The model under review builds one solid part; all positions refer to its coordinate system, in mm. Face numbers are marked on the shaded views. A direction names the side the tool comes from. Give positions to 0.01 mm unless a question says otherwise; leave off trailing zeros. Loops run counter-clockwise (first coordinate to the right, second up) from the corner with the lowest first, then second, coordinate; pieces in that order, holes last. Notation, with made-up numbers: M 20.5,-32.75 L 48.5,-32.75 A22 ccw 48.5,-19.75 Z; hole C -16.5,-23 d7. An arc over 180 degrees is marked long. Return JSON: item names as keys, results as strings.
```python
from build123d import *

# Parameters (mm, degrees)
SKETCH1_R           = 2.5
BOSS_EXTRUDE1_DEPTH = 11
SKETCH2_OUTSIDE_W   = 9.616
SKETCH2_OUTSIDE_H   = 9.616
CUT_EXTRUDE1_DEPTH  = 5
CUT_EXTRUDE2_START  = -5
SKETCH3_R           = 2.5
SKETCH3_R_2         = 1.75
CUT_EXTRUDE2_DEPTH  = 4


with BuildPart() as part:
    # Sketch1 → Boss-Extrude1 (new body)
    with BuildSketch(Plane.XY):
        Circle(SKETCH1_R)
    extrude(amount=BOSS_EXTRUDE1_DEPTH)

    # Sketch2 outside → Cut-Extrude1 (cut)
    with BuildSketch(Plane(origin=(0, 0, 0), x_dir=(-1, 0, 0), z_dir=(0, 0, -1))):
        Rectangle(SKETCH2_OUTSIDE_W, SKETCH2_OUTSIDE_H)
        with BuildLine():
            Line((-1.5, 2), (-1.5, -2))
            ThreePointArc((-1.5, -2), (0, -2.5), (1.5, -2))
            Line((1.5, -2), (1.5, 2))
            ThreePointArc((1.5, 2), (0, 2.5), (-1.5, 2))
        make_face(mode=Mode.SUBTRACT)
    extrude(amount=-CUT_EXTRUDE1_DEPTH, mode=Mode.SUBTRACT)

    # Sketch3 → Cut-Extrude2 (cut)
    with BuildSketch(Plane.XY.offset(11).offset(CUT_EXTRUDE2_START)):
        with Locations(Location((0, 0, 0), (0, 0, 126.869897646))):
            Circle(SKETCH3_R)
        Circle(SKETCH3_R_2, mode=Mode.SUBTRACT)
    extrude(amount=CUT_EXTRUDE2_DEPTH, mode=Mode.SUBTRACT)


solid = part.part
```
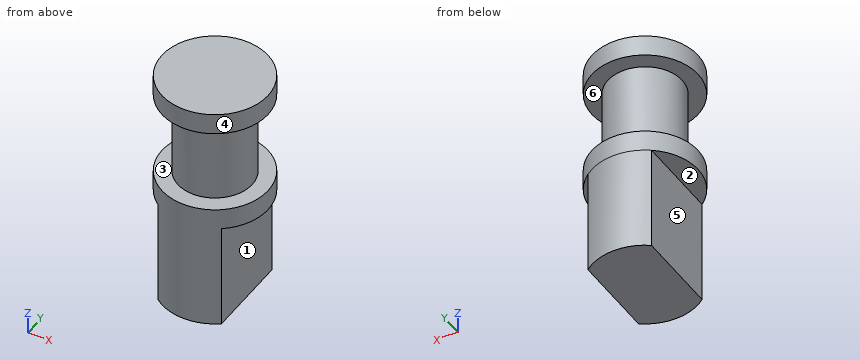
1) Tool access review of the marked faces 4, 5 and 6: name each direction out of +Z, -Z, +X, -X, +Y, -Y from which nothing blocks a thin tool from reaching the whole face with its end or side.
From the geometry:
{"face 4": "+Z, -Z", "face 5": "-Z, -X, +Y, -Y", "face 6": "none"}
2) Consider section B-B on y = 0. Write out the cut boundary in (x, z).
From the geometry:
{"outline": "M -2.5,5 L -1.5,5 L -1.5,0 L 1.5,0 L 1.5,5 L 2.5,5 L 2.5,6 L 1.75,6 L 1.75,10 L 2.5,10 L 2.5,11 L -2.5,11 L -2.5,10 L -1.75,10 L -1.75,6 L -2.5,6 Z"}
3) Consider section A-A on x = -2.05. Write out the cut boundary in (y, z), then the cut area to 3 significant figures.
From the geometry:
{"outline": "M -1.43,5 L 1.43,5 L 1.43,6 L -1.43,6 Z; M -1.43,10 L 1.43,10 L 1.43,11 L -1.43,11 Z", "area": "5.72 mm²"}
4) Consider section D-D on x = 0. Write out the cut boundary in (y, z).
From the geometry:
{"outline": "M -2.5,0 L 2.5,0 L 2.5,6 L 1.75,6 L 1.75,10 L 2.5,10 L 2.5,11 L -2.5,11 L -2.5,10 L -1.75,10 L -1.75,6 L -2.5,6 Z"}
5) Wall thickness on L1, parallel to Z at x = -0.3, y = 2; L2, parallel to Z at x = 2.05, y = 0.4; L3, parallel to X at y = -0.65, z = 3.75: over which ranges is each line inside the solid? List them lowest first. Write a range as from..to.
From the geometry:
{"L1": "0..6, 10..11", "L2": "5..6, 10..11", "L3": "-1.5..1.5"}
6) Insertion check: pin 1 (1.2 mm diameter, centred on y = 1, z = 3.5, fed in from +X); pin 2 (2 mm diameter, centred on y = 1.5, z = 2.5, fed in from -X); pin 3 (0.5 mm diameter, centred on x = 2, y = -1, fed in from -Z). Each pin has a flat end and moves straight along its axis. Give the tip position at first contact, or say it passes through.
From the geometry:
{"pin 1": "x = 1.5", "pin 2": "x = -1.5", "pin 3": "z = 5"}
7) Consider section C-C on y = 2.15. Write out the cut boundary in (x, z).
From the geometry:
{"outline": "M -1.28,0 L 1.28,0 L 1.28,6 L -1.28,6 Z; M -1.28,10 L 1.28,10 L 1.28,11 L -1.28,11 Z"}
8) The part is to be moulded in two halves that separate along Z. For the marked faces 1, 2 and 3, say which applies: released by +Z, released by -Z, zero draft, split by the parting line, or undercut.
From the geometry:
{"face 1": "zero draft", "face 2": "released by -Z", "face 3": "undercut"}
